Geometry check sheet. Reference: drawing and pictorial views, mm from the part's lowest x, y, z. A direction names the side the tool comes from. Round coordinates to 2 decimals unless told otherwise and drop trailing zeros. Order: outer loops, then holes, each group sorted by start corner. A loop starts at its lowest first (then second) coordinate and runs counter-clockwise, first axis right, second up. Notation, with made-up numbers: M 9.5,-5.75 L 39.5,-5.75 A19 ccw 39.5,23.25 Z; hole C 13,-7 d6. An arc over 180 degrees is marked long. Answer as a JSON object with one key per item and string values. Group by question number.
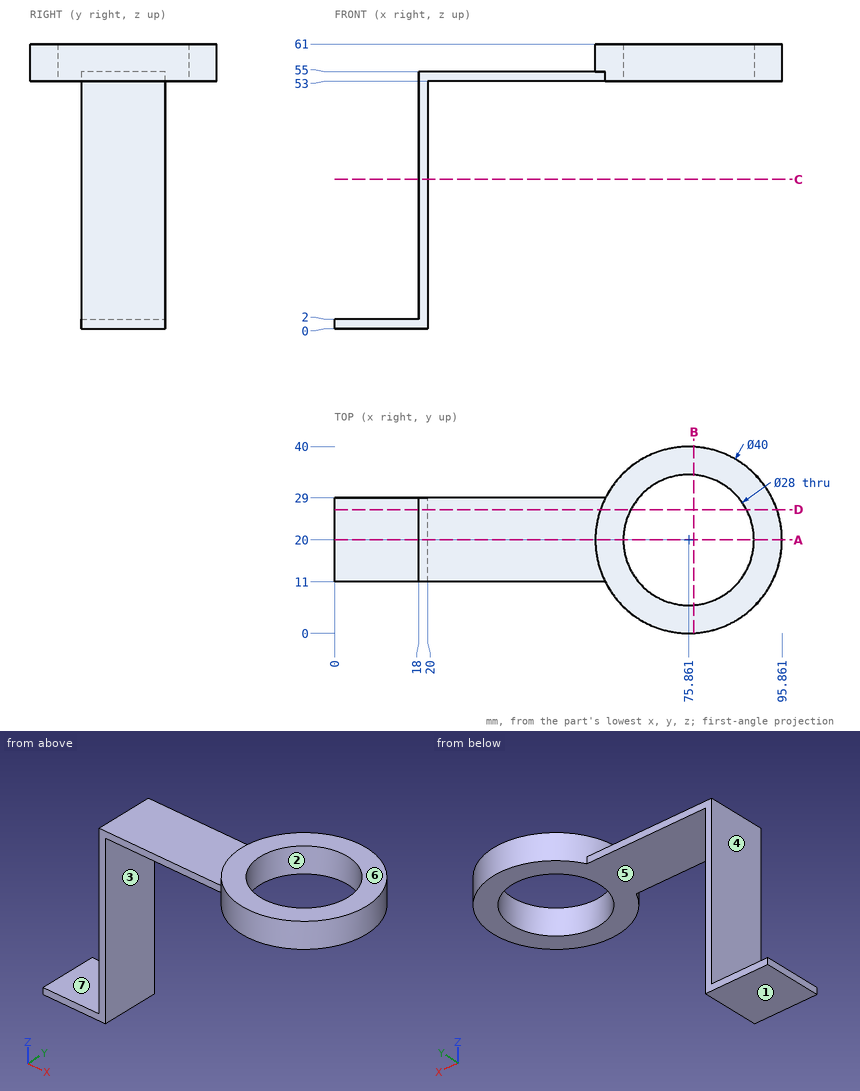
Q1. Cross-section at C-C, the plane z = 32. Record the cut outline in (x, y), then the cut area to 3 significant figures.
Q2. Gauge pin test, flat ends, axial feed: pin 1 Ø20 at (y, z) = (21.5, 22) entering from -X; pin 2 Ø1 at (x, y) = (50, 25) entering from +Z; pin 3 Ø9 at (y, z) = (21, 38.5) entering from +X. Record the tip position at first contact, or that the pin passes through.
Q3. Cross-section at B-B, the plane x = 77. Record the cut outline in (y, z).
Q4. Release check for a two-part mould opening along X. For the marked faces 1, 2, 3 and 4 record: released by +X, released by -X, zero draft, split by the parting line, or undercut.
Q5. Cross-section at D-D, the plane y = 26.5. Record the cut outline in (x, z) (1 decimal), then the cut area to 3 significant figures.
Q6. Cross-section at A-A, the plane y = 20. Record the cut outline in (x, z).
Q7. Tool access check on the marked faces 5, 6 and 7. Record the directions out of +Z, -Z, +X, -X, +Y, -Y that give a thin tool (end or side, any length) a straight path to the whole face; none if there is none.
Q8. Thickness scan on line 1 (X direction, y = 22.5, z = 32); line 2 (Z direction, x = 51, y = 24); line 3 (Z direction, x = 81, y = 35.5). Record the ranges inside material, lowest first. Write a range as from..to.
Conclusion:
{
 "1": {"outline": "M 18,11 L 20,11 L 20,29 L 18,29 Z", "area": "36.0 mm2"},
 "2": {"pin 1": "x = 18", "pin 2": "z = 55", "pin 3": "x = 20"},
 "3": {"outline": "M 0.03,53 L 6.05,53 L 6.05,61 L 0.03,61 Z; M 33.95,53 L 39.97,53 L 39.97,61 L 33.95,61 Z"},
 "4": {"face 1": "zero draft", "face 2": "undercut", "face 3": "released by +X", "face 4": "released by -X"},
 "5": {"outline": "M 0,0 L 20,0 L 20,53 L 63.5,53 L 63.5,61 L 56.9,61 L 56.9,55 L 18,55 L 18,2 L 0,2 Z; M 88.3,53 L 94.8,53 L 94.8,61 L 88.3,61 Z", "area": "324 mm2"},
 "6": {"outline": "M 0,0 L 20,0 L 20,53 L 61.86,53 L 61.86,61 L 55.86,61 L 55.86,55 L 18,55 L 18,2 L 0,2 Z; M 89.86,53 L 95.86,53 L 95.86,61 L 89.86,61 Z"},
 "7": {"face 5": "-Z, +X, +Y, -Y", "face 6": "+Z, +X, -X, +Y, -Y", "face 7": "+Z, -X, +Y, -Y"},
 "8": {"line 1": "18..20", "line 2": "53..55", "line 3": "53..61"}
}
